from build123d import *

# Parameters (mm, degrees)
SKETCH_1_W                   = 150
SKETCH_1_H                   = 75
EXTRUDE_1_DEPTH              = 17
HOLE_WIZARD_M6_1_D           = 6.6
HOLE_WIZARD_M6_1_CBORE_D     = 11
HOLE_WIZARD_M6_1_CBORE_DEPTH = 6.4
SKETCH_8_W                   = 16
SKETCH_8_H                   = 75
EXTRUDE_2_DEPTH              = 75
HOLE_WIZARD_7_0_7_1_D        = 7
SKETCH_11_W                  = 48
SKETCH_11_H                  = 2
CUT_EXTRUDE_1_DEPTH          = 141.406552554
EXTRUDE_3_DEPTH              = 3
CHAMFER_1_SIZE               = 2
SKETCH_13_W                  = 62
SKETCH_13_H                  = 9
CUT_EXTRUDE_2_DEPTH          = 141.406552554
HOLE_WIZARD_7_0_7_2_D        = 7
HOLE_WIZARD_6_0_6_1_D        = 6


with BuildPart() as part:
    # 草图1 → 凸台-拉伸1 (new body)
    with BuildSketch(Plane.XY):
        Rectangle(SKETCH_1_W, SKETCH_1_H)
    extrude(amount=EXTRUDE_1_DEPTH)

    # M6 六角凹头螺钉的柱形沉头孔1 (through all)
    with Locations(Plane.XY.offset(17)):
        with Locations((2.5, 17.5), (-32.5, 17.5), (-32.5, -17.5), (2.5, -17.5)):
            CounterBoreHole(HOLE_WIZARD_M6_1_D / 2, HOLE_WIZARD_M6_1_CBORE_D / 2, HOLE_WIZARD_M6_1_CBORE_DEPTH)

    # 草图8 → 凸台-拉伸2 (add)
    with BuildSketch(Plane.XY.offset(17)):
        with Locations((-57, 0)):
            Rectangle(SKETCH_8_W, SKETCH_8_H)
    extrude(amount=EXTRUDE_2_DEPTH)

    # Ø7.0 (7) 直径孔1 (through all)
    with Locations(Plane(origin=(-49, 0, 0), x_dir=(0, 0, -1), z_dir=(1, 0, 0))):
        with Locations((-75, 31), (-75, -31), (-34, -31), (-34, 31)):
            Hole(HOLE_WIZARD_7_0_7_1_D / 2)

    # 草图11 → 切除-拉伸1 (cut, through all)
    with BuildSketch(Plane.XZ.offset(37.5)):
        with Locations((-15, 1)):
            Rectangle(SKETCH_11_W, SKETCH_11_H)
    extrude(amount=-CUT_EXTRUDE_1_DEPTH, mode=Mode.SUBTRACT)

    # 草图12 → 凸台-拉伸3 (add, symmetric)
    with BuildSketch(Plane(origin=(0, 0, 0), x_dir=(1, 0, 0), z_dir=(0, 1, 0))):
        Polygon((-49, -67), (-39, -67), (-9, -27), (-9, -17), (-39, -17), (-49, -27), align=None)
    extrude(amount=EXTRUDE_3_DEPTH, both=True)

    # 倒角1
    chamfer_1_edges = [part.edges().sort_by_distance(p)[0] for p in [
        (75, -37.5, 8.5),
        (75, 37.5, 8.5),
        (-57, -37.5, 92),
        (-57, 37.5, 92),
        (-75, 37.5, 8.5),
        (-75, -37.5, 8.5),
    ]]
    chamfer(chamfer_1_edges, length=CHAMFER_1_SIZE)

    # 草图13 → 切除-拉伸2 (cut, through all)
    with BuildSketch(Plane.XZ.offset(37.5)):
        with Locations((44, 4.5)):
            Rectangle(SKETCH_13_W, SKETCH_13_H)
    extrude(amount=-CUT_EXTRUDE_2_DEPTH, mode=Mode.SUBTRACT)

    # Ø7.0 (7) 直径孔2 (through all)
    with Locations(Plane.XY.offset(17)):
        with Locations((35, -10), (67, -10)):
            Hole(HOLE_WIZARD_7_0_7_2_D / 2)

    # Ø6.0 (6) 直径孔1 (through all)
    with Locations(Plane.XY.offset(17)):
        with Locations((65, 28.5), (65, 16.5)):
            Hole(HOLE_WIZARD_6_0_6_1_D / 2)


solid = part.part
Model file for the job. Use its own axes, mm. A direction names the side the tool comes from. Coordinates: 2 decimals unless noted, no trailing zeros. Order: outer loops, then holes, each group sorted by start corner. A loop starts at its lowest first (then second) coordinate and runs counter-clockwise, first axis right, second up. Notation, with made-up numbers: M 86,7 L 97,7 A28 cw 97,44 Z; hole C -28.75,-37.75 d2. An arc over 180 degrees is marked long. Return JSON: item names as keys, results as strings.
1. Pull direction X, two halves, no side cores. Call faces 5 (the face through (-44, 0, 22)), 6 (the face through (13, -1, 4)), 7 (the face through (-57.11, 33.95, 76.88)): +X half, -X half, draft (parallel to the pull), parting line (faces both ways), or undercut.
Ans:
{"face 5": "undercut", "face 6": "+X half", "face 7": "draft"}
2. Saw through at C-C (z = 15). Give the number of separate pieces and of enclosed holes in the cut face, and give its area (3 significant figures).
Ans:
{"separate pieces": "1", "enclosed holes": "8", "area": "10,700 mm^2"}
3. Tool access for faces 1 (the face through (-44, 0, 67)), 2 (the face through (5, -20, 10.6)), 3 (the face through (-70, 1, 17)), 4 (the face through (-15, -1, 2)): list every direction of +Z, -Z, +X, -X, +Y, -Y with a clear straight run to the whole face (end or side of a thin tool).
Ans:
{"face 1": "+Z, +X, +Y, -Y", "face 2": "+Z", "face 3": "+Z, -X, +Y, -Y", "face 4": "-Z, +Y, -Y"}
4. Drill centre lines: probe 1 along Y at (x, z) = (-32.5, 15); probe 2 along Y at (x, z) = (-54, 34); probe 3 along Y at (x, z) = (65, 14). Where is each one in solid material? Low to high.
Ans:
{"probe 1": "-37.5 to -23, -12 to 12, 23 to 37.5", "probe 2": "-37.5 to -34.5, -27.5 to 27.5, 34.5 to 37.5", "probe 3": "-37.5 to -12.87, -7.13 to 13.5, 19.5 to 25.5, 31.5 to 37.5"}
5. Flat gauge pins, fed straight in: pin 1 (1.5 mm diameter, centred on y = -11, z = 36.5, fed in from -X); pin 2 (5 mm diameter, centred on y = 0.5, z = 24.5, fed in from +X); pin 3 (12 mm diameter, centred on x = -31, y = -19, fed in from +Z); pin 4 (3.5 mm diameter, centred on x = 65, y = 16.5, fed in from -Z). Where does each tip first touch, or does it go through?
Ans:
{"pin 1": "x = -65", "pin 2": "x = -9", "pin 3": "z = 17", "pin 4": "through"}
6. Saw through at B-B (x = 2.5). Give the cut face in (y, z), and give its area (3 significant figures).
Ans:
{"outline": "M -37.5,2 L -20.8,2 L -20.8,10.6 L -23,10.6 L -23,17 L -37.5,17 Z; M -14.2,2 L 14.2,2 L 14.2,10.6 L 12,10.6 L 12,17 L -12,17 L -12,10.6 L -14.2,10.6 Z; M 20.8,2 L 37.5,2 L 37.5,17 L 23,17 L 23,10.6 L 20.8,10.6 Z", "area": "871 mm^2"}
7. Saw through at D-D (z = 43). Give the cut face in (x, y).
Ans:
{"outline": "M -65,-37.5 L -49,-37.5 L -49,-3 L -21,-3 L -21,3 L -49,3 L -49,37.5 L -65,37.5 Z"}
8. Saw through at A-A (y = -31). Give the cut face in (x, z).
Ans:
{"outline": "M -75,0 L -39,0 L -39,2 L 9,2 L 9,0 L 13,0 L 13,9 L 75,9 L 75,17 L -49,17 L -49,30.5 L -65,30.5 L -65,17 L -75,17 Z; M -65,37.5 L -49,37.5 L -49,71.5 L -65,71.5 Z; M -65,78.5 L -49,78.5 L -49,92 L -65,92 Z"}
